from build123d import *

# Parameters (mm, degrees)
BOSS_EXTRUDE_1_DEPTH = 1050


with BuildPart() as part:
    # Sketch 1 → Boss-Extrude 1 (new, symmetric)
    with BuildSketch(Plane.XY):
        with BuildLine():
            Line((0, 50), (-40, 50))
            ThreePointArc((-40, 50), (-47.071067812, 47.071067812), (-50, 40))
            Line((-50, 40), (-50, 0))
            Line((-50, 0), (-50, -40))
            ThreePointArc((-50, -40), (-47.071067812, -47.071067812), (-40, -50))
            Line((-40, -50), (40, -50))
            ThreePointArc((40, -50), (47.071067812, -47.071067812), (50, -40))
            Line((50, -40), (50, 0))
            Line((50, 0), (50, 40))
            ThreePointArc((50, 40), (47.071067812, 47.071067812), (40, 50))
            Line((40, 50), (0, 50))
        make_face()
        with BuildLine():
            Line((0, 45), (-40, 45))
            ThreePointArc((-40, 45), (-43.535533906, 43.535533906), (-45, 40))
            Line((-45, 40), (-45, 0))
            Line((-45, 0), (-45, -40))
            ThreePointArc((-45, -40), (-43.535533906, -43.535533906), (-40, -45))
            Line((-40, -45), (40, -45))
            ThreePointArc((40, -45), (43.535533906, -43.535533906), (45, -40))
            Line((45, -40), (45, 0))
            Line((45, 0), (45, 40))
            ThreePointArc((45, 40), (43.535533906, 43.535533906), (40, 45))
            Line((40, 45), (0, 45))
        make_face(mode=Mode.SUBTRACT)
    extrude(amount=BOSS_EXTRUDE_1_DEPTH, both=True)


solid = part.part
Verification items for the finished model (mm, model axes). A direction names the side the tool comes from. Coordinates: 2 decimals unless noted, no trailing zeros. Loops run counter-clockwise (first coordinate to the right, second up) from the corner with the lowest first, then second, coordinate; pieces in that order, holes last. Notation, with made-up numbers: (-3.75, -26.5) -> (48.25, -26.5) arc R11 ccw to (48.25, -9.5) -> close; hole circle Ø3 at (81.25, 14). An arc over 180 degrees is marked (long way). Write each question's results on one line, items separated by ' | '.
Item 1: Material ranges on L1, parallel to Y at x = 0, z = -746; L2, parallel to X at y = 43.5, z = 244.5, recorded low to high.
Found:
L1: y = -50 to -45, 45 to 50 | L2: x = -49.37 to -43.57, 43.57 to 49.37
Item 2: Mould release check, pull along X, two halves, no side actions. Record for faces 3 (the face through (-1, -45, 15)), 4 (the face through (1, 50, 15)), 5 (the face through (50, -1, 15)): +X half, -X half, draft (parallel to the pull), parting line (faces both ways), or undercut.
Found:
face 3: undercut | face 4: draft | face 5: +X half
Item 3: Tool access check on faces 1 (the face through (-45, 1, 15)), 2 (the face through (-50, 1, 15)). Record the directions out of +Z, -Z, +X, -X, +Y, -Y that give a thin tool (end or side, any length) a straight path to the whole face; none if there is none.
Found:
face 1: +Z, -Z | face 2: +Z, -Z, -X, +Y, -Y
Item 4: Section check A-A, the plane x = 14.5. Enter the section's corners in (y, z), plus the area to 3 significant figures.
Found:
outline: (-50, -1050) -> (-45, -1050) -> (-45, 1050) -> (-50, 1050) -> close; (45, -1050) -> (50, -1050) -> (50, 1050) -> (45, 1050) -> close | area: 21,000 mm2
Item 5: Section check B-B, the plane z = 264.5. Enter the section's corners in (x, y), plus the area to 3 significant figures.
Found:
outline: (-50, -40) arc R10 ccw to (-40, -50) -> (40, -50) arc R10 ccw to (50, -40) -> (50, 40) arc R10 ccw to (40, 50) -> (-40, 50) arc R10 ccw to (-50, 40) -> close; hole (-45, -40) arc R5 ccw to (-40, -45) -> (40, -45) arc R5 ccw to (45, -40) -> (45, 40) arc R5 ccw to (40, 45) -> (-40, 45) arc R5 ccw to (-45, 40) -> close | area: 1,840 mm2
